Can you work these out from the drawing? Everything is in mm from the part's minimum corner. Coordinates: 2 decimals unless noted, no trailing zeros. Loops run counter-clockwise (first coordinate to the right, second up) from the corner with the lowest first, then second, coordinate; pieces in that order, holes last. Notation, with made-up numbers: (59, 18.25) - (88, 18.25) arc R30 ccw to (88, 56.25) - close; hole circle Ø9 at (-30, 21). An arc over 180 degrees is marked (long way). Put each result on its own line as item: value. Start each with the question number.
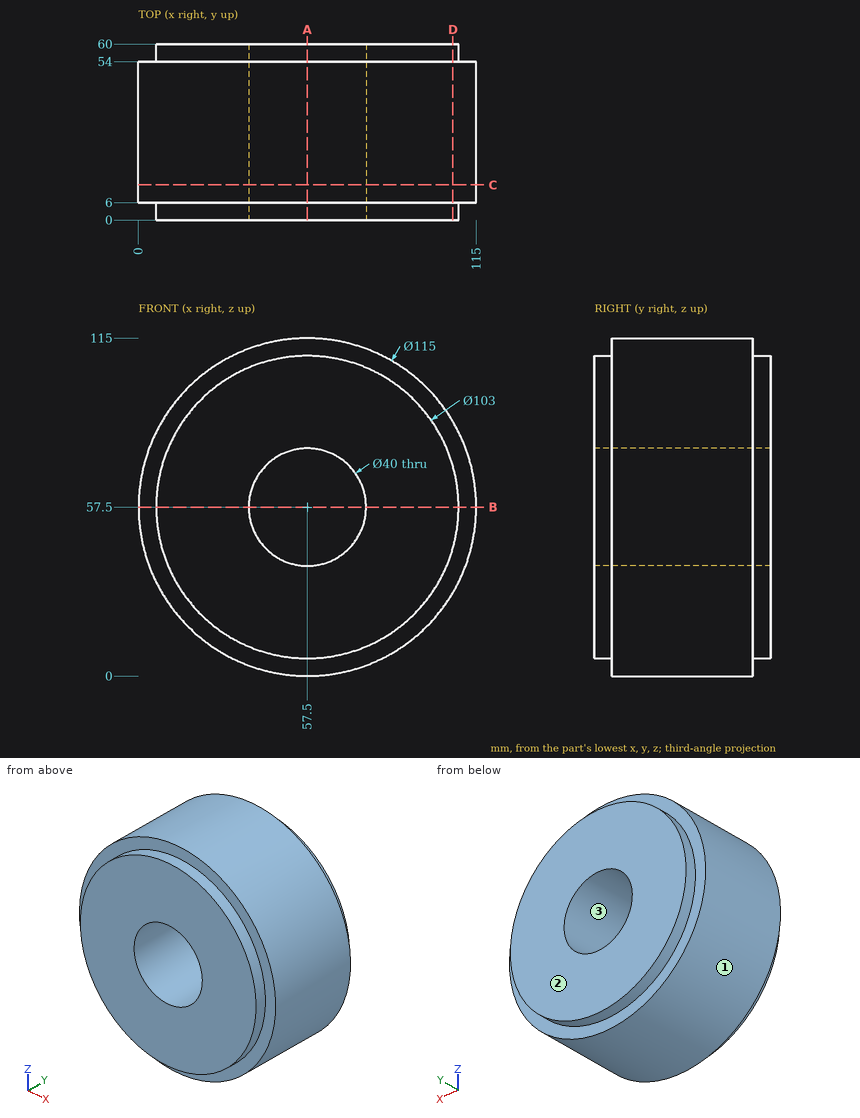
Q1. I want a section at B-B on z = 57.5. List the corners of the cut face in (x, y) for me, and give its area (3 significant figures).
Q2. I want a section at C-C on y = 12. List the corners of the cut face in (x, z) for me.
Q3. Will these pins go through, and if not, where does the flat tip stop? pin 1 (4 mm diameter, centred on x = 38, y = 11.5, fed in from +Z); pin 2 (5 mm diameter, centred on x = 39.5, y = 19.5, fed in from -Z); pin 3 (10 mm diameter, centred on y = 12.5, z = 55.5, fed in from +X); pin 4 (4 mm diameter, centred on x = 52, z = 42, fed in from -Y).
Q4. I want a section at D-D on x = 107. List the corners of the cut face in (y, z) for me.
Q5. Please list where these lines run through material, in increasing order: line 1 along Z through (x, y) = (57, 39.5); line 2 along X through (y, z) = (32, 57.5); line 3 along Y through (x, z) = (107, 76.5). Write a range as [from, to].
Q6. We'd pull the mould along Z, two halves only. Please class the marked faces 1, 2 and 3: released by +Z, released by -Z, zero draft, split by the parting line, or undercut.
Q7. I want a section at A-A on x = 57.5. List the corners of the cut face in (y, z) for me.
Calculated:
1. outline: (0, 6) - (6, 6) - (6, 0) - (37.5, 0) - (37.5, 60) - (6, 60) - (6, 54) - (0, 54) - close; (77.5, 0) - (109, 0) - (109, 6) - (115, 6) - (115, 54) - (109, 54) - (109, 60) - (77.5, 60) - close
1. area: 4,360 mm2
2. outline: circle Ø115 at (57.5, 57.5); hole circle Ø40 at (57.5, 57.5)
3. pin 1: z = 112.27
3. pin 2: z = 2.13
3. pin 3: x = 115
3. pin 4: through
4. outline: (0, 43.29) - (6, 43.29) - (6, 28.24) - (54, 28.24) - (54, 43.29) - (60, 43.29) - (60, 71.71) - (54, 71.71) - (54, 86.76) - (6, 86.76) - (6, 71.71) - (0, 71.71) - close
5. line 1: [0, 37.51], [77.49, 115]
5. line 2: [0, 37.5], [77.5, 115]
5. line 3: [6, 54]
6. face 1: split by the parting line
6. face 2: zero draft
6. face 3: undercut
7. outline: (0, 6) - (6, 6) - (6, 0) - (54, 0) - (54, 6) - (60, 6) - (60, 37.5) - (0, 37.5) - close; (0, 77.5) - (60, 77.5) - (60, 109) - (54, 109) - (54, 115) - (6, 115) - (6, 109) - (0, 109) - close
